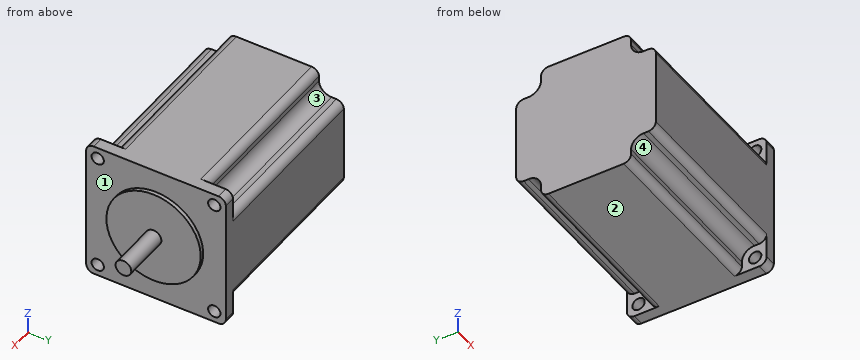
```python
from build123d import *

# Parameters (mm, degrees)
SKETCH_1_W               = 56.4
SKETCH_1_H               = 56.4
EXTRUDE_1_DEPTH          = 76
SKETCH_2_R               = 19.05
EXTRUDE_2_DEPTH          = 1.6
SKETCH_3_R               = 3.175
EXTRUDE_3_DEPTH          = 19.4
FILLET_1_R               = 3
CUT_EXTRUDE_1_DEPTH      = 71.4
SKETCH_5_R               = 2.5
CUT_EXTRUDE_2_DEPTH      = 5
PATTERN_CIRCULAR_3_COUNT = 4
FILLET_2_R               = 3


with BuildPart() as part:
    # 草图1 → 凸台-拉伸1 (new body)
    with BuildSketch(Plane(origin=(0, 0, 0), x_dir=(0, 0, -1), z_dir=(1, 0, 0))):
        Rectangle(SKETCH_1_W, SKETCH_1_H)
    extrude(amount=EXTRUDE_1_DEPTH)

    # 草图2 → 凸台-拉伸2 (add)
    with BuildSketch(Plane(origin=(76, 0, 0), x_dir=(0, 0, -1), z_dir=(1, 0, 0))):
        with Locations(Location((0, 0, 0), (0, 0, 180))):
            Circle(SKETCH_2_R)
    extrude(amount=EXTRUDE_2_DEPTH)

    # 草图3 → 凸台-拉伸3 (add)
    with BuildSketch(Plane(origin=(77.6, 0, 0), x_dir=(0, 0, -1), z_dir=(1, 0, 0))):
        Circle(SKETCH_3_R)
    extrude(amount=EXTRUDE_3_DEPTH)

    # 圆角1
    fillet_1_edges = [part.edges().sort_by_distance(p)[0] for p in [
        (38, -28.2, -28.2),
        (38, -28.2, 28.2),
        (38, 28.2, 28.2),
        (38, 28.2, -28.2),
    ]]
    fillet(fillet_1_edges, radius=FILLET_1_R)

    # 草图4 → 切除-拉伸1 (cut)
    with BuildSketch(Plane.ZY):
        with BuildLine():
            Line((-28.2, 28.2), (-18.2, 28.2))
            Line((-18.2, 28.2), (-18.2, 23.2))
            ThreePointArc((-18.2, 23.2), (-19.664466094, 19.664466094), (-23.2, 18.2))
            Line((-23.2, 18.2), (-28.2, 18.2))
            Line((-28.2, 18.2), (-28.2, 28.2))
        make_face()
    cut_extrude_1 = extrude(amount=-CUT_EXTRUDE_1_DEPTH, mode=Mode.SUBTRACT)

    # 草图5 → 切除-拉伸2 (cut)
    with BuildSketch(Plane.ZY.offset(-71.4)):
        with Locations((-23.55, 23.55)):
            Circle(SKETCH_5_R)
    cut_extrude_2 = extrude(amount=-CUT_EXTRUDE_2_DEPTH, mode=Mode.SUBTRACT)

    # 阵列(圆周)3: 切除-拉伸1, 切除-拉伸2 ×4 about axis
    pattern_circular_3_axis = Axis((0, 0, 0), (1, 0, 0))
    add([cut_extrude_1.rotate(pattern_circular_3_axis, i * 360 / PATTERN_CIRCULAR_3_COUNT) for i in range(1, PATTERN_CIRCULAR_3_COUNT)], mode=Mode.SUBTRACT)
    add([cut_extrude_2.rotate(pattern_circular_3_axis, i * 360 / PATTERN_CIRCULAR_3_COUNT) for i in range(1, PATTERN_CIRCULAR_3_COUNT)], mode=Mode.SUBTRACT)

    # 圆角2
    fillet_2_edges = [part.edges().sort_by_distance(p)[0] for p in [
        (35.7, 28.2, 18.2),
        (35.7, 18.2, 28.2),
        (35.7, 18.2, -28.2),
        (35.7, 28.2, -18.2),
        (35.7, -28.2, -18.2),
        (35.7, -18.2, -28.2),
        (35.7, -18.2, 28.2),
        (35.7, -28.2, 18.2),
    ]]
    fillet(fillet_2_edges, radius=FILLET_2_R)


solid = part.part
```
Can you work these out from the model? Positions are in its coordinate system, mm. Face numbers are marked on the shaded views. A direction names the side the tool comes from. Give positions to 0.01 mm unless a question says otherwise; leave off trailing zeros. Loops run counter-clockwise (first coordinate to the right, second up) from the corner with the lowest first, then second, coordinate; pieces in that order, holes last. Notation, with made-up numbers: M -11,-33.75 L -6,-33.75 A30 ccw -6,-2.75 Z; hole C 61,29 d2. An arc over 180 degrees is marked long. Use CSV: the item, a comma, the result in double quotes. Start each with the question number.
1. If I drill on L1, parallel to Y at x = 73, z = -23; L2, parallel to X at y = 3.5, z = 12, over which ranges is the centre line in solid material (lowest first)?
2. For P1, Ø2, axis at y = -10, z = 6.5, coming from the +X side; P2, Ø1.6, axis at x = 44.5, y = 24.5, coming from the -Z side; P3, Ø0.6, axis at x = 40, y = -24, coming from the +Z side, each with a flat end and sliding along its axis, tell me the tip position at first contact or that it passes through.
3. Imagine slicing it at C-C, the plane y = 14. Write out the boundary of the cut face in (x, z), plus the area to 3 significant figures.
4. Imagine slicing it at A-A, the plane x = 30. Write out the boundary of the cut face in (y, z), plus the area to 3 significant figures.
5. Imagine slicing it at D-D, the plane z = -16.5. Write out the boundary of the cut face in (x, y), plus the area to 3 significant figures.
6. On a 3-axis mill with a long thin cutter (end or side, diameter ignored), from which of +Z, -Z, +X, -X, +Y, -Y can I reach the whole of each face in a straight line? I mean the marked faces 1, 2, 3 and 4. Say none if no direction works.
7. Imagine slicing it at B-B, the plane z = 0. Write out the boundary of the cut face in (x, y) (3 decimals).
Response values:
1,L1,"-28.2 to -25.99, -21.11 to 21.11, 25.99 to 28.2"
1,L2,"0 to 77.6"
2,P1,"x = 77.6"
2,P2,"z = -18.2"
2,P3,"z = 18.2"
3,outline,"M 0,-28.2 L 76,-28.2 L 76,-12.92 L 77.6,-12.92 L 77.6,12.92 L 76,12.92 L 76,28.2 L 0,28.2 Z"
3,area,"4,330 mm^2"
4,outline,"M -28.2,-15.2 A3 ccw -25.2,-18.2 L -23.2,-18.2 A5 cw -18.2,-23.2 L -18.2,-25.2 A3 ccw -15.2,-28.2 L 15.2,-28.2 A3 ccw 18.2,-25.2 L 18.2,-23.2 A5 cw 23.2,-18.2 L 25.2,-18.2 A3 ccw 28.2,-15.2 L 28.2,15.2 A3 ccw 25.2,18.2 L 23.2,18.2 A5 cw 18.2,23.2 L 18.2,25.2 A3 ccw 15.2,28.2 L -15.2,28.2 A3 ccw -18.2,25.2 L -18.2,23.2 A5 cw -23.2,18.2 L -25.2,18.2 A3 ccw -28.2,15.2 Z"
4,area,"2,790 mm^2"
5,outline,"M 0,-27.9 L 71.4,-27.9 L 71.4,-28.2 L 76,-28.2 L 76,-9.52 L 77.6,-9.52 L 77.6,9.52 L 76,9.52 L 76,28.2 L 71.4,28.2 L 71.4,27.9 L 0,27.9 Z"
5,area,"4,270 mm^2"
6,face 1,"+X"
6,face 2,"-Z, +X, -X, +Y, -Y"
6,face 3,"+Z, -X, +Y"
6,face 4,"-Z, -X, -Y"
7,outline,"M 0,-28.2 L 76,-28.2 L 76,-19.05 L 77.6,-19.05 L 77.6,-3.175 L 97,-3.175 L 97,3.175 L 77.6,3.175 L 77.6,19.05 L 76,19.05 L 76,28.2 L 0,28.2 Z"
